from build123d import *

# Parameters (mm, degrees)
BASE_BLOCK_SKETCH_W           = 92
BASE_BLOCK_SKETCH_H           = 32
BASE_BLOCK_DEPTH              = 48
MOUNTING_FLANGE_SKETCH_W      = 48
MOUNTING_FLANGE_SKETCH_H      = 12.000000000000002
MOUNTING_FLANGE_DEPTH         = 29
FLANGE_HOLES_SKETCH_R         = 2.999999999999994
FLANGE_HOLES_SKETCH_R_2       = 2.9999999999999947
FLANGE_HOLES_2X_DEPTH         = 29
UPRIGHT_LUG_DEPTH             = 16
UPRIGHT_LUG_CHAMFER_CUT_DEPTH = 16
SIDE_LUG_DEPTH                = 16
SIDE_LUG_CHAMFER_CUT_DEPTH    = 16
UPRIGHT_LUG_HOLE_SKETCH_R     = 3.0000000000000018
UPRIGHT_LUG_HOLE_SKETCH_R_2   = 3.000000000000001
UPRIGHT_LUG_HOLE_DEPTH        = 16
HUB_BODY_DEPTH                = 35
HUB_START                     = 3
HUB_COLLAR_SKETCH_R           = 20.5
HUB_COLLAR_41_DEPTH           = 3
HUB_BORE_SKETCH_R             = 13.999999999999996
HUB_BORE_28_DEPTH             = 38
ANGLED_RELIEF_CUT_30DEG_DEPTH = 38
RELIEF_POCKET_DEPTH           = 38
SPOT_FACE_SKETCH_R            = 12.500000000000002
SPOT_FACE_RECESS_DEPTH        = 2
THROUGH_HOLE_SKETCH_R         = 6.000000000000003
THROUGH_HOLE_12_DEPTH         = 30
ARM_BLOCK_SKETCH_W            = 12.999999999999993
ARM_BLOCK_SKETCH_H            = 19.000000000000004
ARM_BLOCK_DEPTH               = 19
CLAMP_LUG_DEPTH               = 20
CLAMP_PAD_DEPTH               = 1
CLAMP_HOLE_SKETCH_R           = 3.0000000000000004
CLAMP_HOLE_6_DEPTH            = 20
HUB_SLOT_CUT_DEPTH            = 20


with BuildPart() as part:
    # Base Block Sketch → Base Block (new body)
    with BuildSketch(Plane.XY):
        with Locations((46, 16)):
            Rectangle(BASE_BLOCK_SKETCH_W, BASE_BLOCK_SKETCH_H)
    extrude(amount=BASE_BLOCK_DEPTH)

    # Mounting Flange Sketch → Mounting Flange (add)
    with BuildSketch(Plane(origin=(92, 0, 0), x_dir=(0, 0, -1), z_dir=(1, 0, 0))):
        with Locations((-24, 16)):
            Rectangle(MOUNTING_FLANGE_SKETCH_W, MOUNTING_FLANGE_SKETCH_H)
    extrude(amount=MOUNTING_FLANGE_DEPTH)

    # Flange Holes Sketch → Flange Holes 2x (cut)
    with BuildSketch(Plane.XZ.offset(-9.999999999999998)):
        with Locations(Location((106.5, 13, 0), (0, 0, 270))):
            Circle(FLANGE_HOLES_SKETCH_R)
        with Locations(Location((106.5, 34.99999999999999, 0), (0, 0, 270))):
            Circle(FLANGE_HOLES_SKETCH_R_2)
    extrude(amount=-FLANGE_HOLES_2X_DEPTH, mode=Mode.SUBTRACT)

    # Upright Lug Sketch → Upright Lug (add)
    with BuildSketch(Plane.XZ):
        Polygon((38, 0), (62, 0), (78, 0), (78, 16), (62, 16), (38, 16), align=None)
    extrude(amount=UPRIGHT_LUG_DEPTH)

    # Upright Lug Chamfer Sketch → Upright Lug Chamfer Cut (cut)
    with BuildSketch(Plane.XY.offset(16)):
        Polygon((78, -16), (62, -16), (78, 0), align=None)
    extrude(amount=-UPRIGHT_LUG_CHAMFER_CUT_DEPTH, mode=Mode.SUBTRACT)

    # Side Lug Sketch → Side Lug (add)
    with BuildSketch(Plane(origin=(0, 32, 0), x_dir=(1, 0, 0), z_dir=(0, 1, 0))):
        Polygon((38, 0), (62, 0), (78, 0), (78, -16), (62, -16), (38, -16), align=None)
    extrude(amount=SIDE_LUG_DEPTH)

    # Side Lug Chamfer Sketch → Side Lug Chamfer Cut (cut)
    with BuildSketch(Plane.XY.offset(16)):
        Polygon((78, 48), (62, 48), (78, 32), align=None)
    extrude(amount=-SIDE_LUG_CHAMFER_CUT_DEPTH, mode=Mode.SUBTRACT)

    # Upright Lug Hole Sketch → Upright Lug Hole (cut)
    with BuildSketch(Plane.XY.offset(16)):
        with Locations((50, 40)):
            Circle(UPRIGHT_LUG_HOLE_SKETCH_R)
        with Locations((50, -8)):
            Circle(UPRIGHT_LUG_HOLE_SKETCH_R_2)
    extrude(amount=-UPRIGHT_LUG_HOLE_DEPTH, mode=Mode.SUBTRACT)

    # Hub Body Sketch → Hub Body (add)
    with BuildSketch(Plane.XZ):
        with BuildLine():
            ThreePointArc((3.3573e-13, 27.379229861405094), (21.334077351297417, 25.748287751556113), (32.5, 43.99999999999999))
            ThreePointArc((32.5, 44), (32.4012544943822, 46.009680336633146), (32.10596926288294, 48.00000000000083))
            Line((32.10596926288278, 48), (0, 48))
            Line((0, 48), (0, 27.379229861404976))
        make_face()
        with BuildLine():
            Line((0, 48), (32.10596926288278, 48))
            ThreePointArc((32.10596926288294, 48.00000000000083), (0.9216100131877187, 61.24874706464494), (3.3573e-13, 27.379229861405094))
            Line((0, 27.379229861404976), (0, 48))
        make_face()
    extrude(amount=-HUB_BODY_DEPTH)

    # Hub Collar Sketch → Hub Collar _41 (add)
    with BuildSketch(Plane.XZ.offset(HUB_START)):
        with Locations(Location((11.999999999999998, 44, 0), (0, 0, 270))):
            Circle(HUB_COLLAR_SKETCH_R)
    extrude(amount=-HUB_COLLAR_41_DEPTH)

    # Hub Bore Sketch → Hub Bore _28 (cut)
    with BuildSketch(Plane.XZ.offset(3)):
        with Locations(Location((11.999999999999998, 44, 0), (0, 0, 270))):
            Circle(HUB_BORE_SKETCH_R)
    extrude(amount=-HUB_BORE_28_DEPTH, mode=Mode.SUBTRACT)

    # Angled Relief Sketch → Angled Relief Cut 30deg (cut)
    with BuildSketch(Plane.XZ):
        Polygon((69.03034488539707, 29.00000000000001), (79.99999999999999, 48), (38.10596926288314, 48), (38.1059692628831, 29), (67.89066123526882, 29), align=None)
    extrude(amount=-ANGLED_RELIEF_CUT_30DEG_DEPTH, mode=Mode.SUBTRACT)

    # Relief Pocket Sketch → Relief Pocket (cut)
    with BuildSketch(Plane.XZ):
        with BuildLine():
            Line((32.052589846453245, 39.74046476127714), (32.021949545440904, 34.99941169508152))
            ThreePointArc((32.021949545440904, 34.99941169508152), (33.74970667402833, 30.786581192003514), (37.93792982799573, 29.00000000000004))
            Line((37.93792982799573, 29), (38.1059692628831, 29))
            Line((38.1059692628831, 29), (38.10596926288314, 48))
            Line((38.10596926288314, 48), (32.1059692628831, 48))
            ThreePointArc((32.10596926288309, 48), (32.499571898565115, 43.8675161309467), (32.0525898464532, 39.74046476127714))
        make_face()
    extrude(amount=-RELIEF_POCKET_DEPTH, mode=Mode.SUBTRACT)

    # Spot Face Sketch → Spot Face Recess (cut)
    with BuildSketch(Plane.XY.offset(29)):
        with Locations((53.48413735669789, 16)):
            Circle(SPOT_FACE_SKETCH_R)
    extrude(amount=-SPOT_FACE_RECESS_DEPTH, mode=Mode.SUBTRACT)

    # Through Hole Sketch → Through Hole _12 (cut)
    with BuildSketch(Plane.XY.offset(27.000000000000004)):
        with Locations((53.48413735669789, 16)):
            Circle(THROUGH_HOLE_SKETCH_R)
    extrude(amount=-THROUGH_HOLE_12_DEPTH, mode=Mode.SUBTRACT)

    # Arm Block Sketch → Arm Block (add)
    with BuildSketch(Plane(origin=(12, 0, 0), x_dir=(0, 0, -1), z_dir=(1, 0, 0))):
        with Locations((-58, 16)):
            Rectangle(ARM_BLOCK_SKETCH_W, ARM_BLOCK_SKETCH_H)
    extrude(amount=-ARM_BLOCK_DEPTH)

    # Clamp Lug Sketch → Clamp Lug (add)
    with BuildSketch(Plane.XZ.offset(-6.499999999999999)):
        with BuildLine():
            Line((-6.999999999999999, 51.69740215917034), (-37, 51.69740215917034))
            Line((-37, 51.69740215917034), (-37, 38.697402159170345))
            Line((-37, 38.697402159170345), (-3.229691527211141, 30.277518592251866))
            ThreePointArc((-3.229691527211141, 30.277518592251866), (-8.189621059274332, 40.446241217681404), (-6.999999999999999, 51.69740215917034))
        make_face()
    extrude(amount=-CLAMP_LUG_DEPTH)

    # Clamp Pad Sketch → Clamp Pad (add)
    with BuildSketch(Plane(origin=(0, 25.5, 0), x_dir=(1, 0, 0), z_dir=(0, 1, 0))):
        with BuildLine():
            Line((-6.999999999999999, -51.69740215917034), (-6.999999999999999, -64.5))
            Line((-6.999999999999999, -64.5), (11.999999999999998, -64.5))
            ThreePointArc((11.999999999999998, -64.5), (0.5445808514701636, -61.00068740173455), (-6.999999999999999, -51.69740215917034))
        make_face()
    extrude(amount=CLAMP_PAD_DEPTH)

    # Clamp Hole Sketch → Clamp Hole _6 (cut)
    with BuildSketch(Plane.XY.offset(64.5)):
        with Locations(Location((12, 16.5, 0), (0, 0, 90))):
            Circle(CLAMP_HOLE_SKETCH_R)
    extrude(amount=-CLAMP_HOLE_6_DEPTH, mode=Mode.SUBTRACT)

    # Hub Slot Sketch → Hub Slot Cut (cut)
    with BuildSketch(Plane.XZ.offset(-6.499999999999999)):
        with BuildLine():
            Line((12, 51.50000000000001), (12, 57.99999999999999))
            ThreePointArc((12, 57.99999999999999), (5.254631218383986, 56.26784414638529), (0.17840958246311683, 51.50000000000001))
            Line((0.17840958246311683, 51.50000000000001), (12, 51.50000000000001))
        make_face()
    extrude(amount=-HUB_SLOT_CUT_DEPTH, mode=Mode.SUBTRACT)


solid = part.part
CAD build for the part. Positions are in the model's coordinates, mm. A direction names the side the tool comes from. Give positions to 0.01 mm unless a question says otherwise; leave off trailing zeros. Loops run counter-clockwise (first coordinate to the right, second up) from the corner with the lowest first, then second, coordinate; pieces in that order, holes last. Notation, with made-up numbers: M 11,22.25 L 52,22.25 A34 ccw 52,60.25 Z; hole C -25,75.5 d7. An arc over 180 degrees is marked long. Answer in a Markdown table with one row per item. Add a question column.
Item 1: Probe probe 1 along Z at (x, y) = (12, 8); probe 2 along Z at (x, y) = (105, 14); probe 3 along X at (y, z) = (29, 36). List the from-to ranges inside material, lowest first.
Item 2: Band-saw the part on B-B on z = 45. Give the cut face in (x, y).
Item 3: Band-saw the part on A-A on y = 40. Give the cut face in (x, z).
Item 4: Band-saw the part on C-C on y = 16. Give the cut face in (x, z).
Item 5: Band-saw the part on D-D on x = 50. Give the cut face in (y, z).
Item 6: Tool access for faces 5 (the face through (-2, 6.5, 61)), 6 (the face through (28.81, 15.73, 55.73)), 7 (the face through (65.03, 11.21, 28.01)): list every direction of +Z, -Z, +X, -X, +Y, -Y with a clear straight run to the whole face (end or side of a thin tool).
Item 7: Mould opens along Z. For faces 1 (the face through (54, -8, 16)), 2 (the face through (46, 16, 0)), 3 (the face through (121, 16, 24)), 4 (the face through (33.704, 15.776, 30.833)) say: +Z half, -Z half, draft (parallel to the pull), parting line (faces both ways), or undercut.
Item 8: Drop flat-ended pins along their axis: P1, Ø8, axis at y = -5, z = 9.5, coming from the -X side; P2, Ø8, axis at y = 25.5, z = 13.5, coming from the +X side; P3, Ø1, axis at x = 89.5, z = 12.5, coming from the +Y side; P4, Ø6, axis at y = 37, z = 28, coming from the -X side. Give the stop position or say it passes through.
Reply:
| question | item | result |
|---|---|---|
| 1 | probe 1 | z = 0 to 30, 58 to 64.5 |
| 1 | probe 2 | z = 0 to 10.4, 15.6 to 32.4, 37.6 to 48 |
| 1 | probe 3 | x = -6.87 to 0.51, 23.49 to 32.03, 73.07 to 92 |
| 2 | outline | M -37,6.5 L -8.48,6.5 L -8.48,-3 L -1.96,-3 L -1.96,35 L -8.48,35 L -8.48,26.5 L -37,26.5 Z; M 25.96,-3 L 32.48,-3 L 32.48,35 L 25.96,35 Z; M 78.27,0 L 92,0 L 92,10 L 121,10 L 121,22 L 92,22 L 92,32 L 78.27,32 Z |
| 3 | outline | M 38,0 L 47,0 L 47,16 L 38,16 Z; M 53,0 L 70,0 L 70,16 L 53,16 Z |
| 4 | outline | M -37,38.7 L -3.23,30.28 A20.5 ccw 0,27.38 L 0,0 L 47.48,0 L 47.48,27 L 40.98,27 L 40.98,29 L 37.94,29 A6 cw 32.02,35 L 32.05,39.74 A20.5 ccw 14.96,64.29 L 14.96,57.68 A14 cw long 9.04,57.68 L 9.04,64.5 L -7,64.5 L -7,51.7 L -37,51.7 Z; M 59.48,0 L 121,0 L 121,48 L 80,48 L 69.03,29 L 65.98,29 L 65.98,27 L 59.48,27 Z; hole C 106.5,13 d6; hole C 106.5,35 d6 |
| 5 | outline | M -16,0 L -11,0 L -11,16 L -16,16 Z; M -5,0 L 11.12,0 L 11.12,27 L 4,27 L 4,29 L 0,29 L 0,16 L -5,16 Z; M 20.88,0 L 37,0 L 37,16 L 32,16 L 32,29 L 28,29 L 28,27 L 20.88,27 Z; M 43,0 L 48,0 L 48,16 L 43,16 Z |
| 6 | face 5 | +Z, -X, -Y |
| 6 | face 6 | none |
| 6 | face 7 | +Z |
| 7 | face 1 | +Z half |
| 7 | face 2 | -Z half |
| 7 | face 3 | draft |
| 7 | face 4 | undercut |
| 8 | P1 | stops at x = 38 |
| 8 | P2 | stops at x = 121 |
| 8 | P3 | stops at y = 32 |
| 8 | P4 | stops at x = -3.19 |
